from build123d import *

# Parameters (mm, degrees)
EXTRUDE_1_DEPTH = 5


with BuildPart() as part:
    # 草图1 → 凸台-拉伸1 (new, symmetric)
    with BuildSketch(Plane.XY):
        with BuildLine():
            Line((-50, 33), (50, 33))
            ThreePointArc((50, 33), (83, 0), (50, -33))
            Line((50, -33), (-50, -33))
            ThreePointArc((-50, -33), (-83, 0), (-50, 33))
        make_face()
        with BuildLine():
            Line((-50, 30), (50, 30))
            ThreePointArc((50, 30), (80, 0), (50, -30))
            Line((50, -30), (-50, -30))
            ThreePointArc((-50, -30), (-80, 0), (-50, 30))
        make_face(mode=Mode.SUBTRACT)
    extrude(amount=EXTRUDE_1_DEPTH, both=True)


solid = part.part
Design review of the part built by this model. Coordinates are the model's own, in mm. A direction names the side the tool comes from. Give positions to 0.01 mm unless a question says otherwise; leave off trailing zeros. Order: outer loops, then holes, each group sorted by start corner. A loop starts at its lowest first (then second) coordinate and runs counter-clockwise, first axis right, second up.
1. Add section C-C, the plane x = 3.5. State the section outline as (y, z) points, then the cut area to 3 significant figures.
Solution:
outline: (-33, -5) - (-30, -5) - (-30, 5) - (-33, 5) - close; (30, -5) - (33, -5) - (33, 5) - (30, 5) - close
area: 60.0 mm2
2. Add section A-A, the plane y = 0. State the section outline as (x, z) points.
Solution:
outline: (-83, -5) - (-80, -5) - (-80, 5) - (-83, 5) - close; (80, -5) - (83, -5) - (83, 5) - (80, 5) - close
3. Tool access review of faces 1 (the cylindrical face through (79.993, 0.66, 0.07)), 2 (the flat face through (1, -33, 0)): name each direction out of +Z, -Z, +X, -X, +Y, -Y from which nothing blocks a thin tool from reaching the whole face with its end or side.
Solution:
face 1: +Z, -Z
face 2: +Z, -Z, +X, -X, -Y
4. To check wall thickness, follow L1, parallel to Y at x = 14, z = -3.25; L2, parallel to X at y = 1.5, z = 1.75; L3, parallel to X at y = -22, z = 3.5. State the ranges of each line that lie inside material, in increasing order.
Solution:
L1: y = -33 to -30, 30 to 33
L2: x = -82.97 to -79.96, 79.96 to 82.97
L3: x = -74.6 to -70.4, 70.4 to 74.6
5. Mouldability with a two-part tool opening along Y and no side actions: class faces 3 (the cylindrical face through (-79.993, -0.66, 0.07)), 4 (the cylindrical face through (82.99, 0.73, 0.07)), 5 (the flat face through (7, 32, 5)) as +Y half, -Y half, draft (parallel to the pull), parting line (faces both ways), or undercut.
Solution:
face 3: undercut
face 4: parting line
face 5: draft
6. Add section B-B, the plane z = 3.25. State the section outline as (x, y) points.
Solution:
outline: (-50, -33) - (50, -33) arc R33 ccw to (50, 33) - (-50, 33) arc R33 ccw to start; hole (-50, -30) - (50, -30) arc R30 ccw to (50, 30) - (-50, 30) arc R30 ccw to start
7. For pin 1 Ø1 at (y, z) = (-1, 3.5) entering from +X; pin 2 Ø1 at (y, z) = (-17, 0) entering from +X, all flat-tipped, find the tip position at first contact; note any pin that passes through.
Solution:
pin 1: stops at x = 83
pin 2: stops at x = 78.58
